Can you work these out from the drawing? Everything is in mm from the part's minimum corner. Give positions to 0.01 mm unless a question says otherwise; leave off trailing zeros. Loops run counter-clockwise (first coordinate to the right, second up) from the corner with the lowest first, then second, coordinate; pieces in that order, holes last. Notation, with made-up numbers: M 2,84 L 23,84 A20 ccw 23,92 Z; hole C 37.5,-14 d2. An arc over 180 degrees is marked long. Use CSV: the item, a comma, the result in double quotes.
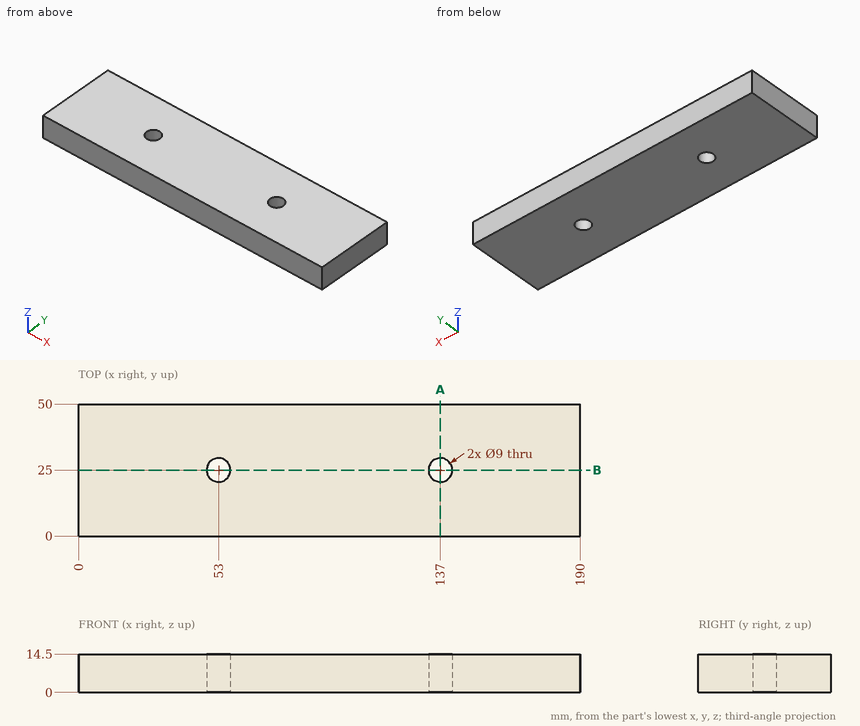
Q1. I want a section at B-B, the plane y = 25. Please give me the cut outline in (x, z), then the cut area to 3 significant figures.
Model answer:
outline,"M 0,0 L 48.5,0 L 48.5,14.5 L 0,14.5 Z; M 57.5,0 L 132.5,0 L 132.5,14.5 L 57.5,14.5 Z; M 141.5,0 L 190,0 L 190,14.5 L 141.5,14.5 Z"
area,"2,490 mm2"
Q2. I'm going to push a flat-ended pin straight in: P1, Ø8, axis at x = 137, y = 25, coming from the -Z side (3 decimals). Where does the tip first touch, or does it pass through?
Model answer:
P1,"through"
Q3. Please list where these lines run through material, in increasing order: L1, parallel to X at y = 25, z = 10.5; L2, parallel to Y at x = 53, z = 11.5; L3, parallel to Y at x = 54.5, z = 13. Write a range as from..to.
Model answer:
L1,"0..48.5, 57.5..132.5, 141.5..190"
L2,"0..20.5, 29.5..50"
L3,"0..20.76, 29.24..50"
Q4. I want a section at A-A, the plane x = 137. Please give me the cut outline in (y, z), then the cut area to 4 significant figures.
Model answer:
outline,"M 0,0 L 20.5,0 L 20.5,14.5 L 0,14.5 Z; M 29.5,0 L 50,0 L 50,14.5 L 29.5,14.5 Z"
area,"594.5 mm2"
